from build123d import *

# Parameters (mm, degrees)
CLEARANCE_HOLE_FOR_M1_62_D = 1.8


with BuildPart() as part:
    # Sketch1 → Revolution1 (revolve)
    with BuildSketch(Plane.XY, mode=Mode.PRIVATE) as revolution1_sk:
        with BuildLine():
            Line((0, -15.453508628), (-15, -15.453508628))
            Line((-15, -15.453508628), (-11.121601357, -13.029509476))
            ThreePointArc((-11.121601357, -13.029509476), (-10.994443143, -12.972884255), (-10.856601887, -12.953508628))
            Line((-10.856601887, -12.953508628), (-8, -12.953508628))
            Line((-8, -12.953508628), (-8, -11.453508628))
            Line((-8, -11.453508628), (-8, -9.453508628))
            Line((-8, -9.453508628), (0, -9.453508628))
            Line((0, -9.453508628), (0, -15.453508628))
        make_face()
    revolve(revolution1_sk.sketch.rotate(Axis((0, 20.85946169, 0), (0, -1, 0)), 270), axis=Axis((0, 20.85946169, 0), (0, -1, 0)))

    # Clearance hole for M1.62 (through all)
    with Locations(Plane(origin=(0, -15.453508628, 0), x_dir=(-1, 0, 0), z_dir=(0, -1, 0))):
        with Locations((0, 0)):
            Hole(CLEARANCE_HOLE_FOR_M1_62_D / 2)


solid = part.part
Geometry: final body of the model. Coordinates: model frame, mm. A direction names the side the tool comes from. Round coordinates to 2 decimals unless told otherwise and drop trailing zeros. Loops run counter-clockwise (first coordinate to the right, second up) from the corner with the lowest first, then second, coordinate; pieces in that order, holes last. Notation, with made-up numbers: M 53,33 L 87,33 A14 ccw 87,52 Z; hole C -2.5,33.5 d8. An arc over 180 degrees is marked long. Put each result on its own line as item: value. Start each with the question number.
(1) Section query A-A (x = 0). Return loops of the section in (y, z).
(2) Set-up query: faces 1 (the face through (0, -15.454, -3)), 2 (the face through (7.2, -12.954, -4.1)). Return all of +Z, -Z, +X, -X, +Y, -Y with unobstructed straight access to the full face (end or side cutting, diameter ignored); none if empty.
(3) Draft query along Z for faces 3 (the face through (7.81, -11.18, -1.73)), 4 (the face through (0, -9.454, 2)), 5 (the face through (0.86, -12.41, -0.27)). Return one class per face: +Z half, -Z half, draft (parallel to the pull), parting line (faces both ways), or undercut.
(4) Section query D-D (y = -14.75). Return loops of the section in (x, z), then the cut area to 3 significant figures.
(5) Material intervals for line 1 along Y through (x, z) = (10.5, 2.75); line 2 along Z through (x, y) = (-3.5, -11); line 3 along X through (y, z) = (-14.5, 9), sorted ascending. Write a range as [from, to].
(6) Section query C-C (y = -12). Return loops of the section in (x, z), then the cut area to 3 significant figures.
(7) Section query B-B (z = 0). Return loops of the section in (x, y), then the cut area to 3 significant figures.
(8) Contact query for flat-ended pins moving along their axis: pin 1 Ø1 at (x, z) = (10.5, 9) entering from +Y; pin 2 Ø2 at (x, z) = (-1.5, -9.5) entering from +Y. Output: stop coordinate, or through.
Findings below:
1. outline: M -15.45,-15 L -13.03,-11.12 A0.5 ccw -12.95,-10.86 L -12.95,-8 L -9.45,-8 L -9.45,-0.9 L -15.45,-0.9 Z; M -15.45,0.9 L -9.45,0.9 L -9.45,8 L -12.95,8 L -12.95,10.86 A0.5 ccw -13.03,11.12 L -15.45,15 Z
2. face 1: +Z, -Z, +X, -X, -Y
2. face 2: +Y
3. face 3: parting line
3. face 4: draft
3. face 5: undercut
4. outline: C 0,0 d27.75; hole C 0,0 d1.8
4. area: 602 mm2
5. line 1: y = [-15.45, -12.95]
5. line 2: z = [-7.19, 7.19]
5. line 3: x = [-10.03, 10.03]
6. outline: C 0,0 d16; hole C 0,0 d1.8
6. area: 199 mm2
7. outline: M -15,-15.45 L -0.9,-15.45 L -0.9,-9.45 L -8,-9.45 L -8,-12.95 L -10.86,-12.95 A0.5 ccw -11.12,-13.03 Z; M 0.9,-15.45 L 15,-15.45 L 11.12,-13.03 A0.5 ccw 10.86,-12.95 L 8,-12.95 L 8,-9.45 L 0.9,-9.45 Z
7. area: 110 mm2
8. pin 1: stops at y = -14.41
8. pin 2: stops at y = -12.95
